For this review, use the dimensioned drawing (mm, ordinates from the lowest corner) and the shaded views. Coordinates: 2 decimals unless noted, no trailing zeros. Loops run counter-clockwise (first coordinate to the right, second up) from the corner with the lowest first, then second, coordinate; pieces in that order, holes last.
1. Take a section at A-A, the plane x = 25. State the section outline as (y, z) points, then the cut area to 4 significant figures.
2. Take a section at C-C, the plane z = 42. State the section outline as (x, y) points, then the cut area to 3 significant figures.
3. To check wall thickness, follow probe 1 along Z at (x, y) = (15.5, 36.5); probe 2 along X at (y, z) = (2, 156); probe 3 along X at (y, z) = (37.5, 320). State the ranges of each line that lie inside material, in increasing order.
4. Take a section at D-D, the plane x = 45. State the section outline as (y, z) points, then the cut area to 3 significant figures.
5. Clearance check with flat-ended pins moving along their axes: P1, Ø1.5, axis at y = 15, z = 367, coming from the -X side; P2, Ø6, axis at y = 14, z = 180.5, coming from the +X side; P3, Ø3, axis at y = 39.5, z = 400.5, coming from the +X side. State where each tip first meets the part, or that it passes through.
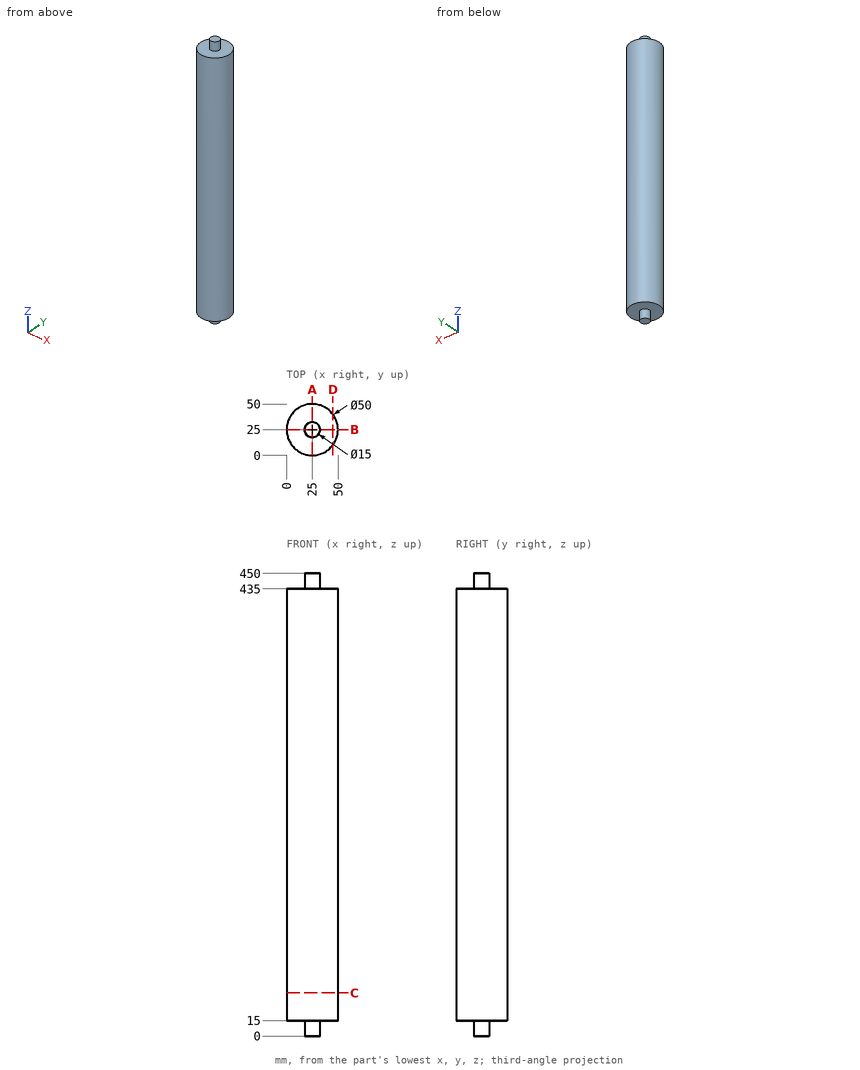
Results list:
1. outline: (0, 15) - (17.5, 15) - (17.5, 0) - (32.5, 0) - (32.5, 15) - (50, 15) - (50, 435) - (32.5, 435) - (32.5, 450) - (17.5, 450) - (17.5, 435) - (0, 435) - close
1. area: 21,450 mm2
2. outline: circle Ø50 at (25, 25)
2. area: 1,960 mm2
3. probe 1: z = 15 to 435
3. probe 2: x = 15.2 to 34.8
3. probe 3: x = 3.35 to 46.65
4. outline: (10, 15) - (40, 15) - (40, 435) - (10, 435) - close
4. area: 12,600 mm2
5. P1: stops at x = 1.77
5. P2: stops at x = 48.69
5. P3: stops at x = 46.35
